Read the model definition and answer for the solid it produces. Units are mm, in the model's axes. Coordinates: 2 decimals unless noted, no trailing zeros. Write each loop counter-clockwise with the first axis right and the second up, starting at its lowest first coordinate (ties: lowest second). Pieces come first, ordered by that corner, then holes. Notation, with made-up numbers: (-24, 57.5) -> (-6, 57.5) arc R23 cw to (-6, 83.5) -> close; hole circle Ø4 at (16, 47). An arc over 180 degrees is marked (long way). One line per item, written item: value. Start each with the question number.
1. Find section B-B, the plane x = 180. Write down the section's boundary in (y, z), and give its area (3 significant figures).
2. Find section A-A, the plane y = 0. Write down the section's boundary in (x, z), and give its area (3 significant figures).
3. Consider line 1 along Y through (x, z) = (180, 14.75); line 2 along X through (y, z) = (8.5, 17); line 3 along X through (y, z) = (5.5, 11.5). Determine where each line is inside the solid, lowest interval first.
4. For a pull along X with two mould halves and no side action, classify faces 1 (the flat face through (448, 0, 10)), 2 (the cylindrical face through (435.522, 8.475, 9.86)), 3 (the cylindrical face through (183.815, 1.201, 9.86)), 4 (the flat face through (264, 20, 10)) as pulls with the +X half, pulls with the -X half, needs draft (parallel to the pull), parting line crosses it, or undercut.
```python
from build123d import *

# Parameters (mm, degrees)
SKETCH_2_W          = 400
SKETCH_2_H          = 40
SKETCH_2_R          = 4
EXTRUDE_1_DEPTH     = 20
SKETCH_4_W          = 20
SKETCH_4_H          = 40
EXTRUDE_2_DEPTH     = 248
HOLE_WIZARD_M10_1_D = 8.5
SKETCH_9_W          = 20
SKETCH_9_H          = 40
CUT_EXTRUDE_2_DEPTH = 285


with BuildPart() as part:
    # 草图2 → 凸台-拉伸1 (new body)
    with BuildSketch(Plane.XY):
        Rectangle(SKETCH_2_W, SKETCH_2_H)
        with Locations((180, 0)):
            Circle(SKETCH_2_R, mode=Mode.SUBTRACT)
    extrude(amount=EXTRUDE_1_DEPTH)

    # 草图4 → 凸台-拉伸2 (add)
    with BuildSketch(Plane(origin=(200, 0, 0), x_dir=(0, 0, -1), z_dir=(1, 0, 0))):
        with Locations((-10, 0)):
            Rectangle(SKETCH_4_W, SKETCH_4_H)
    extrude(amount=EXTRUDE_2_DEPTH)

    # M10 螺纹孔1 (through all)
    with Locations(Plane.XY.offset(20)):
        with Locations((431.276, 8.288)):
            Hole(HOLE_WIZARD_M10_1_D / 2)

    # 草图9 → 切除-拉伸2 (cut)
    with BuildSketch(Plane.ZY.offset(200)):
        with Locations((10, 0)):
            Rectangle(SKETCH_9_W, SKETCH_9_H)
    extrude(amount=-CUT_EXTRUDE_2_DEPTH, mode=Mode.SUBTRACT)


solid = part.part
```
Answer block:
1. outline: (-20, 0) -> (-4, 0) -> (-4, 20) -> (-20, 20) -> close; (4, 0) -> (20, 0) -> (20, 20) -> (4, 20) -> close
1. area: 640 mm2
2. outline: (85, 0) -> (176, 0) -> (176, 20) -> (85, 20) -> close; (184, 0) -> (448, 0) -> (448, 20) -> (184, 20) -> close
2. area: 7,100 mm2
3. line 1: y = -20 to -4, 4 to 20
3. line 2: x = 85 to 427.03, 435.52 to 448
3. line 3: x = 85 to 428.07, 434.48 to 448
4. face 1: pulls with the +X half
4. face 2: undercut
4. face 3: undercut
4. face 4: needs draft
